from build123d import *

# Parameters (mm, degrees)
BOSS_EXTRUDE1_DEPTH = 8
SKETCH2_R           = 4.25
CUT_EXTRUDE1_DEPTH  = 10
CUT_EXTRUDE3_DEPTH  = 10
CIRPATTERN1_COUNT   = 3
SKETCH4_R           = 2.1
CUT_EXTRUDE4_DEPTH  = 33.3190556
CIRPATTERN2_COUNT   = 3
SKETCH6_R           = 2.15
CUT_EXTRUDE6_DEPTH  = 10


with BuildPart() as part:
    # Sketch1 → Boss-Extrude1 (new body)
    with BuildSketch(Plane(origin=(0, 0, 0), x_dir=(1, 0, 0), z_dir=(0, 1, 0))):
        Polygon((0, 23.094010768), (-20, 11.547005384), (-20, -11.547005384), (0, -23.094010768), (20, -11.547005384), (20, 11.547005384), align=None)
    extrude(amount=BOSS_EXTRUDE1_DEPTH)

    # Sketch2 → Cut-Extrude1 (cut)
    with BuildSketch(Plane(origin=(0, 8, 0), x_dir=(1, 0, 0), z_dir=(0, 1, 0))):
        with Locations(Location((0, 0, 0), (0, 0, 270))):
            Circle(SKETCH2_R)
    extrude(amount=-CUT_EXTRUDE1_DEPTH, mode=Mode.SUBTRACT)

    # Sketch3 → Cut-Extrude3 (cut)
    with BuildSketch(Plane(origin=(0, 8, 0), x_dir=(1, 0, 0), z_dir=(0, 1, 0))):
        Polygon((-9.133974596, 17.820508076), (-10.866025404, 16.820508076), (-5.866025404, 8.160254038), (-4.133974596, 9.160254038), align=None)
    cut_extrude3 = extrude(amount=-CUT_EXTRUDE3_DEPTH, mode=Mode.SUBTRACT)

    # CirPattern1: Cut-Extrude3 ×3 about axis
    cirpattern1_axis = Axis((0, 0, 0), (0, 1, 0))
    for i in range(1, CIRPATTERN1_COUNT):
        add(cut_extrude3.rotate(cirpattern1_axis, i * 360 / CIRPATTERN1_COUNT), mode=Mode.SUBTRACT)

    # Sketch4 → Cut-Extrude4 (cut, symmetric)
    with BuildSketch(Plane.XY.offset(-1)):
        with Locations((16, 4)):
            Circle(SKETCH4_R)
    cut_extrude4 = extrude(amount=CUT_EXTRUDE4_DEPTH, both=True, mode=Mode.SUBTRACT)

    # CirPattern2: Cut-Extrude4 ×3 about axis
    cirpattern2_axis = Axis((0, -2, 0), (0, 1, 0))
    for i in range(1, CIRPATTERN2_COUNT):
        add(cut_extrude4.rotate(cirpattern2_axis, i * 360 / CIRPATTERN2_COUNT), mode=Mode.SUBTRACT)

    # Sketch6 → Cut-Extrude6 (cut)
    with BuildSketch(Plane(origin=(-14.906511483, 7, 5.40190095), x_dir=(1, 0, 0), z_dir=(0, 1, 0))):
        with Locations((10.906511483, 12.330104181)):
            Circle(SKETCH6_R)
        with Locations(Location((18.906511483, -1.52630228, 0), (0, 0, 270))):
            Circle(SKETCH6_R)
    extrude(amount=-CUT_EXTRUDE6_DEPTH, mode=Mode.SUBTRACT)


solid = part.part
CAD build for the part. Positions are in the model's coordinates, mm. A direction names the side the tool comes from. Give positions to 0.01 mm unless a question says otherwise; leave off trailing zeros. Write each loop counter-clockwise with the first axis right and the second up, starting at its lowest first coordinate (ties: lowest second). Pieces come first, ordered by that corner, then holes. Notation, with made-up numbers: (74, 0) -> (92, 0) arc R26 ccw to (92, 16) -> close; hole circle Ø8 at (18.25, 89). An arc over 180 degrees is marked (long way). Return JSON: item names as keys, results as strings.
Item 1: Band-saw the part on C-C (x = 1). Give the number of separate pieces and of enclosed holes in the cut face, then the cut area to 3 significant figures.
Answer below:
{"separate pieces": "2", "enclosed holes": "2", "area": "262 mm2"}
Item 2: Two-plate mould, pull along X, no slides. Class faces 5 (the cylindrical face through (-13.872, 4.092, -8.043)), 6 (the flat face through (9.86, 3.94, 17.4)), 7 (the flat face through (-15.497, 3.944, 14.147)): +X half, -X half, draft (parallel to the pull), parting line (faces both ways), or undercut.
Answer below:
{"face 5": "undercut", "face 6": "+X half", "face 7": "-X half"}
Item 3: Band-saw the part on A-A (z = -1.5). List the corners of the cut face in (x, y), then the cut area to 3 significant figures.
Answer below:
{"outline": "(-20, 0) -> (-3.98, 0) -> (-3.98, 8) -> (-20, 8) -> close; (3.98, 0) -> (20, 0) -> (20, 8) -> (3.98, 8) -> close; hole circle Ø4.2 at (16, 4)", "area": "243 mm2"}
Item 4: Band-saw the part on B-B (x = 17). List the corners of the cut face in (y, z), then the cut area to 3 significant figures.
Answer below:
{"outline": "(0, -13.28) -> (2.15, -13.28) -> (2.15, -1) -> (0, -1) -> close; (0, 1) -> (2.15, 1) -> (2.15, 13.28) -> (0, 13.28) -> close; (5.85, -13.28) -> (8, -13.28) -> (8, -1) -> (5.85, -1) -> close; (5.85, 1) -> (8, 1) -> (8, 13.28) -> (5.85, 13.28) -> close", "area": "106 mm2"}
Item 5: Tool access for faces 1 (the flat face through (4, 7, 7)), 2 (the cylindrical face through (-14.044, 4.092, 7.944)), 3 (the flat face through (14, 2, -1)), 4 (the flat face through (-7.845, 2.278, -11.589)): list every direction of +Z, -Z, +X, -X, +Y, -Y with a clear straight run to the whole face (end or side of a thin tool).
Answer below:
{"face 1": "-Y", "face 2": "none", "face 3": "+X, +Y, -Y", "face 4": "+Y, -Y"}
Item 6: Drop flat-ended pins along their axis: pin 1 (1.3 mm diameter, centred on x = 4.5, z = 6, fed in from -Y); pin 2 (1.5 mm diameter, centred on y = 7, z = -13, fed in from -X); pin 3 (1 mm diameter, centred on y = 5, z = 0, fed in from +X). Give the stop position or say it passes through.
Answer below:
{"pin 1": "stops at y = 7", "pin 2": "stops at x = -18.78", "pin 3": "stops at x = 10"}
Item 7: Drill centre lines: probe 1 along Z at (x, y) = (-12, 5.5); probe 2 along Y at (x, z) = (16, 11.5); probe 3 along Z at (x, y) = (-5.5, 2.5). Where is each one in solid material? Low to high.
Answer below:
{"probe 1": "z = -16.17 to -13.24, -9.85 to 9.85, 13.24 to 16.17", "probe 2": "y = 0 to 1.9, 6.1 to 8", "probe 3": "z = -19.92 to -17, -13.6 to -11.53, -5.39 to 8.37, 11.53 to 13.6, 17 to 19.92"}
